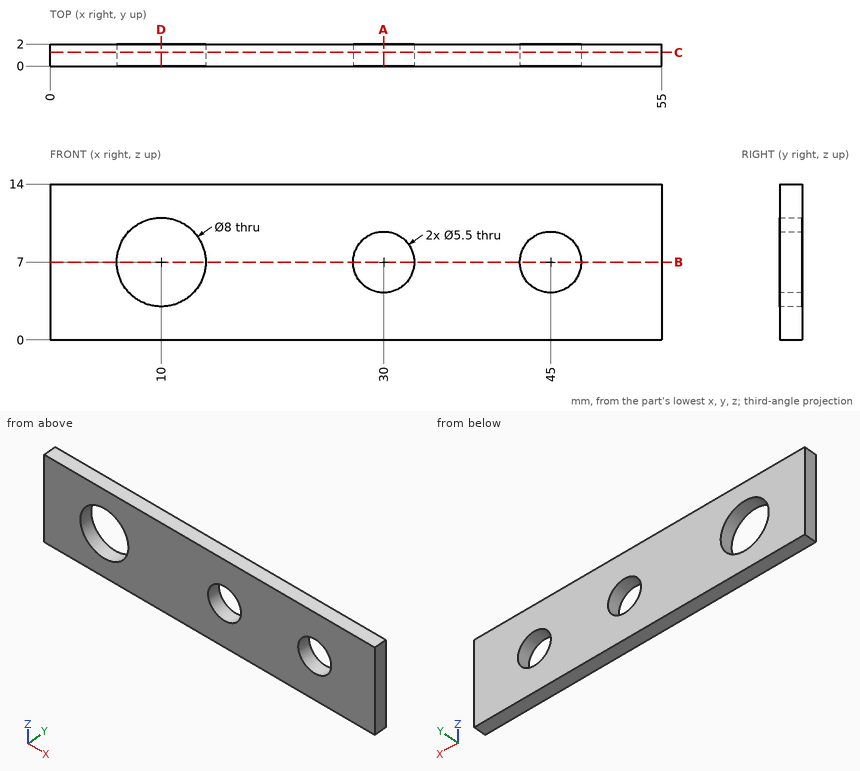
The figure shows three views and two pictorial views of one solid part (mm, origin at its lowest corner). Answer the questions. Coordinates: 2 decimals unless noted, no trailing zeros. Loops run counter-clockwise (first coordinate to the right, second up) from the corner with the lowest first, then second, coordinate; pieces in that order, holes last. Notation, with made-up numbers: (64, 18.5) -> (97, 18.5) arc R30 ccw to (97, 53.5) -> close; hole circle Ø4 at (4, -35.5). An arc over 180 degrees is marked (long way). Use one line per item in the form item = value. Start each with the question number.
Item 1: The part is cut by section C-C on y = 1.25. Determine the outline of the cut face in (x, z).
Item 2: The part is cut by section D-D on x = 10. Determine the outline of the cut face in (y, z), then the cut area to 3 significant figures.
Item 3: The part is cut by section A-A on x = 30. Determine the outline of the cut face in (y, z).
Item 4: Consider L1, parallel to X at y = 1.3, z = 7; L2, parallel to X at y = 0.3, z = 8.5; L3, parallel to Z at x = 44, y = 0.45. Determine where each line is inside the solid, lowest interval first. Write a range as [from, to].
Item 5: The part is cut by section B-B on z = 7. Determine the outline of the cut face in (x, y), then the cut area to 3 significant figures.
Item 6: A flat-ended cylindrical pin translates along its axis: pin 1 Ø4.5 at (x, z) = (30, 7) entering from -Y. Find the tip coordinate at first contact, or state that the pin passes through.
Answer key:
q1.outline = (0, 0) -> (55, 0) -> (55, 14) -> (0, 14) -> close; hole circle Ø8 at (10, 7); hole circle Ø5.5 at (30, 7); hole circle Ø5.5 at (45, 7)
q2.outline = (0, 0) -> (2, 0) -> (2, 3) -> (0, 3) -> close; (0, 11) -> (2, 11) -> (2, 14) -> (0, 14) -> close
q2.area = 12.0 mm2
q3.outline = (0, 0) -> (2, 0) -> (2, 4.25) -> (0, 4.25) -> close; (0, 9.75) -> (2, 9.75) -> (2, 14) -> (0, 14) -> close
q4.L1 = [0, 6], [14, 27.25], [32.75, 42.25], [47.75, 55]
q4.L2 = [0, 6.29], [13.71, 27.7], [32.3, 42.7], [47.3, 55]
q4.L3 = [0, 4.44], [9.56, 14]
q5.outline = (0, 0) -> (6, 0) -> (6, 2) -> (0, 2) -> close; (14, 0) -> (27.25, 0) -> (27.25, 2) -> (14, 2) -> close; (32.75, 0) -> (42.25, 0) -> (42.25, 2) -> (32.75, 2) -> close; (47.75, 0) -> (55, 0) -> (55, 2) -> (47.75, 2) -> close
q5.area = 72.0 mm2
q6.pin_1 = through
